from build123d import *

# Parameters (mm, degrees)
BASE_BRACKET_DEPTH    = 50
PIVOT_LUG_DEPTH       = 13
PIVOT_HOLE_SKETCH_R   = 9.5
PIVOT_HOLE_19_DEPTH   = 13
GUSSET_DEPTH          = 30
GUSSET_TRIM_CUT_DEPTH = 20


with BuildPart() as part:
    # Base Profile Sketch → Base Bracket (new body)
    with BuildSketch(Plane.XY):
        Polygon((0, 0), (16, 0), (100, 0), (100, 10), (16, 10), (16, 56), (0, 56), align=None)
    extrude(amount=BASE_BRACKET_DEPTH)

    # Pivot Lug Sketch → Pivot Lug (add)
    with BuildSketch(Plane(origin=(100, 0, 0), x_dir=(0, 0, -1), z_dir=(1, 0, 0))):
        with BuildLine():
            Line((0, -54), (0, 10))
            Line((0, 10), (-50, 10))
            Line((-50, 10), (-83.040714674, -21.181904589))
            ThreePointArc((-83.040714674, -21.181904589), (-87.657063924, -42.016273484), (-70, -54))
            Line((-70, -54), (0, -54))
        make_face()
    extrude(amount=-PIVOT_LUG_DEPTH)

    # Pivot Hole Sketch → Pivot Hole Ø19 (cut)
    with BuildSketch(Plane(origin=(100, 0, 0), x_dir=(0, 0, -1), z_dir=(1, 0, 0))):
        with Locations((-70, -35)):
            Circle(PIVOT_HOLE_SKETCH_R)
    extrude(amount=-PIVOT_HOLE_19_DEPTH, mode=Mode.SUBTRACT)

    # Gusset Sketch → Gusset (add)
    with BuildSketch(Plane.XY.offset(50)):
        Polygon((16, 56), (16, 10), (87, 10), align=None)
    extrude(amount=-GUSSET_DEPTH)

    # Gusset Trim Sketch → Gusset Trim Cut (cut)
    with BuildSketch(Plane.XY.offset(50)):
        Polygon((16, 56), (16, 10), (87, 10), align=None)
    extrude(amount=-GUSSET_TRIM_CUT_DEPTH, mode=Mode.SUBTRACT)


solid = part.part
Work out the finished part from the listing and answer in its coordinate system (mm). A direction names the side the tool comes from. Give positions to 0.01 mm unless a question says otherwise; leave off trailing zeros. Order: outer loops, then holes, each group sorted by start corner. A loop starts at its lowest first (then second) coordinate and runs counter-clockwise, first axis right, second up. Notation, with made-up numbers: (-6, 61) -> (31, 61) arc R25 ccw to (31, 92) -> close; hole circle Ø11 at (-19.75, 84.25). An arc over 180 degrees is marked (long way). Answer as a JSON object with one key per item and string values. Group by question number.
1. Consider line 1 along X through (y, z) = (-40, 25); line 2 along Z through (x, y) = (47.5, 22.5); line 3 along Y through (x, z) = (92, 70). Determine where each line is inside the solid, lowest interval first. Write a range as [from, to].
2. Section C-C on z = 11 is taken. Determine the outline of the cut face in (x, y).
3. Section B-B on z = 68.5 is taken. Determine the outline of the cut face in (x, y), plus the area to 3 significant figures.
4. A tool of negligible diameter and unlimited length cuts with its end or side. For faces 4 (the flat face through (16, 33, 10)), 5 (the flat face through (43, 0, 25)), 6 (the flat face through (100, -22, 35)), 7 (the flat face through (59, 10, 19)), 8 (the flat face through (35, 23, 30)), from which of +Z, -Z, +X, -X, +Y, -Y can it reach the whole face along a straight path? Write none if from no direction.
5. Section A-A on y = -35 is taken. Determine the outline of the cut face in (x, z).
6. Section D-D on x = 88.5 is taken. Determine the outline of the cut face in (y, z).
7. The mould has two halves that part along Z. Classify faces 1 (the flat face through (23.6, 9.7, 50)), 2 (the flat face through (0, 28, 25)), 3 (the cylindrical face through (93.591, -32.146, 60.939)): released by +Z, released by -Z, zero draft, split by the parting line, or undercut.
8. Flat-ended cylindrical pins translate along their axes: pin 1 Ø22 at (y, z) = (39, 6) entering from +X; pin 2 Ø19 at (y, z) = (-13, 61.5) entering from -X; pin 3 Ø5 at (x, y) = (56, 24) entering from +Z. Find the tip coordinate at first contact, or state that the pin passes through.
Result sheet:
{
 "1": {"line 1": "x = [87, 100]", "line 2": "z = [20, 30]", "line 3": "y = [-54, -44.5], [-25.5, -8.87]"},
 "2": {"outline": "(0, 0) -> (87, 0) -> (87, -54) -> (100, -54) -> (100, 10) -> (16, 10) -> (16, 56) -> (0, 56) -> close"},
 "3": {"outline": "(87, -54) -> (100, -54) -> (100, -44.38) -> (87, -44.38) -> close; (87, -25.62) -> (100, -25.62) -> (100, -7.46) -> (87, -7.46) -> close", "area": "361 mm^2"},
 "4": {"face 4": "-Z, +X, +Y", "face 5": "+Z, -Z, -X, -Y", "face 6": "+Z, -Z, +X, +Y, -Y", "face 7": "+X, +Y", "face 8": "+Z, +X, +Y"},
 "5": {"outline": "(87, 0) -> (100, 0) -> (100, 60.5) -> (87, 60.5) -> close; (87, 79.5) -> (100, 79.5) -> (100, 89) -> (87, 89) -> close"},
 "6": {"outline": "(-54, 0) -> (10, 0) -> (10, 50) -> (-21.18, 83.04) arc R19 ccw to (-54, 70) -> close; hole circle Ø19 at (-35, 70)"},
 "7": {"face 1": "released by +Z", "face 2": "zero draft", "face 3": "undercut"},
 "8": {"pin 1": "stops at x = 16", "pin 2": "stops at x = 87", "pin 3": "stops at z = 30"}
}
